Verification items for the finished model (mm, model axes). A direction names the side the tool comes from. Give positions to 0.01 mm unless a question says otherwise; leave off trailing zeros. Write each loop counter-clockwise with the first axis right and the second up, starting at its lowest first coordinate (ties: lowest second). Pieces come first, ordered by that corner, then holes. Notation, with made-up numbers: M 2.25,-10 L 50.25,-10 A34 cw 50.25,23 Z; hole C 30.5,-33.5 d2. An arc over 180 degrees is marked long. Answer as a JSON object with one key per item and string values.
```python
from build123d import *

# Parameters (mm, degrees)
SKETCH_2_R               = 6.25
CUT_EXTRUDE_1_DEPTH      = 140.896390232
PATTERN_CIRCULAR_1_COUNT = 6
SKETCH_3_R               = 27.5
CUT_EXTRUDE_2_DEPTH      = 140.896390232
CUT_EXTRUDE_START        = -15
CUT_EXTRUDE_3_DEPTH      = 15
PATTERN_CIRCULAR_2_COUNT = 6
PATTERN_CIRCULAR_3_COUNT = 6


with BuildPart() as part:
    # 草图1 → 旋转1 (revolve)
    with BuildSketch(Plane.XY, mode=Mode.PRIVATE) as revolve_1_sk:
        Polygon((0, 0), (0, 95), (30, 95), (30, 50), (39, 50), (39, 35), (30, 35), (30, 0), align=None)
    revolve(revolve_1_sk.sketch.rotate(Axis((0, 0, 0), (1, 0, 0)), 90), axis=Axis((0, 0, 0), (1, 0, 0)))

    # 草图2 → 切除-拉伸1 (cut, through all)
    with BuildSketch(Plane.ZY):
        with Locations((0, 80)):
            Circle(SKETCH_2_R)
    cut_extrude_1 = extrude(amount=-CUT_EXTRUDE_1_DEPTH, mode=Mode.SUBTRACT)

    # 阵列(圆周)1: 切除-拉伸1 ×6 about axis
    pattern_circular_1_axis = Axis((0, 0, 0), (1, 0, 0))
    for i in range(1, PATTERN_CIRCULAR_1_COUNT):
        add(cut_extrude_1.rotate(pattern_circular_1_axis, i * 360 / PATTERN_CIRCULAR_1_COUNT), mode=Mode.SUBTRACT)

    # 草图3 → 切除-拉伸2 (cut, through all)
    with BuildSketch(Plane.ZY):
        Circle(SKETCH_3_R)
    extrude(amount=-CUT_EXTRUDE_2_DEPTH, mode=Mode.SUBTRACT)

    # 草图6 → 切除-拉伸3 (cut)
    with BuildSketch(Plane.ZY.offset(CUT_EXTRUDE_START)):
        with BuildLine():
            Line((-16, 80), (-16, 93.642938869))
            ThreePointArc((-16, 93.642938869), (0, 95), (16, 93.642938869))
            Line((16, 93.642938869), (16, 80))
            ThreePointArc((16, 80), (0, 64), (-16, 80))
        make_face()
    cut_extrude_3 = extrude(amount=CUT_EXTRUDE_3_DEPTH, mode=Mode.SUBTRACT)

    # 阵列(圆周)2: 切除-拉伸3 ×6 about axis
    pattern_circular_2_axis = Axis((0, 0, 0), (1, 0, 0))
    for i in range(1, PATTERN_CIRCULAR_2_COUNT):
        add(cut_extrude_3.rotate(pattern_circular_2_axis, i * 360 / PATTERN_CIRCULAR_2_COUNT), mode=Mode.SUBTRACT)

    # 草图8 → M12 螺纹孔1 (revolve, cut)
    with BuildSketch(Plane(origin=(0, 69.282032303, 40), x_dir=(0, 0, 1), z_dir=(0, 1, 0))):
        Polygon((0, 0), (0, 21.064389157), (5.1, 18), (5.1, 0), align=None)
    hole_wizard_m12_1 = revolve(axis=Axis((-6.35, 69.282032303, 40), (1, 0, 0)), mode=Mode.SUBTRACT)

    # 阵列(圆周)3: M12 螺纹孔1 ×6 about axis
    pattern_circular_3_axis = Axis((0, 0, 0), (1, 0, 0))
    for i in range(1, PATTERN_CIRCULAR_3_COUNT):
        add(hole_wizard_m12_1.rotate(pattern_circular_3_axis, i * 360 / PATTERN_CIRCULAR_3_COUNT), mode=Mode.SUBTRACT)


solid = part.part
```
1) Section check C-C on z = 22.5. Record the boundary of the cut face in (x, y).
Completed:
{"outline": "M 0,-92.3 L 30,-92.3 L 30,-44.65 L 39,-44.65 L 39,-26.81 L 30,-26.81 L 30,-15.81 L 0,-15.81 Z; M 0,15.81 L 30,15.81 L 30,26.81 L 39,26.81 L 39,44.65 L 30,44.65 L 30,92.3 L 0,92.3 Z"}
2) Go/stop test with flat-tipped pins: pin 1 (18 mm diameter, centred on y = -45, z = -62.5, fed in from -X); pin 2 (15 mm diameter, centred on x = 7, y = -83.5, fed in from -Z); pin 3 (4 mm diameter, centred on x = 18.5, y = -29.5, fed in from +Z); pin 4 (1.5 mm diameter, centred on x = 29, z = 48, fed in from +Y). Record where each tip stops, or that it passes through.
Completed:
{"pin 1": "stops at x = 0", "pin 2": "stops at z = -57", "pin 3": "stops at z = 90.93", "pin 4": "stops at y = 82.42"}
3) Access from +Z, -Z, +X, -X, +Y, -Y to the whole of each face (thin tool, end or side, straight path). Record for faces 5 (the face through (7.6, -29.6, -83.27)), 6 (the face through (7.605, -57.315, 67.272)), 7 (the face through (30, 18, -21)), 8 (the face through (15, -43, 75)).
Completed:
{"face 5": "-X, -Y", "face 6": "+Z, -X", "face 7": "+X", "face 8": "-X"}
4) Release check for a two-part mould opening along Y. For faces 1 (the face through (15, 87, 0)), 2 (the face through (15, -43, -75)), 3 (the face through (7.6, 32.31, -55.25)), 4 (the face through (7.6, 29.51, -83.11)) record: pulls with the +Y half, pulls with the -Y half, needs draft (parallel to the pull), parting line crosses it, or undercut.
Completed:
{"face 1": "needs draft", "face 2": "undercut", "face 3": "undercut", "face 4": "pulls with the +Y half"}
5) Section check A-A on z = 0. Record the boundary of the cut face in (x, y).
Completed:
{"outline": "M 0,-64 L 15,-64 L 15,-73.75 L 30,-73.75 L 30,-50 L 39,-50 L 39,-35 L 30,-35 L 30,-27.5 L 0,-27.5 Z; M 0,27.5 L 30,27.5 L 30,35 L 39,35 L 39,50 L 30,50 L 30,73.75 L 15,73.75 L 15,64 L 0,64 Z; M 15,-95 L 30,-95 L 30,-86.25 L 15,-86.25 Z; M 15,86.25 L 30,86.25 L 30,95 L 15,95 Z"}
6) Section check D-D on x = 5. Count the separate pieces of the cut face and the enclosed holes in it, and give its area (3 significant figures).
Completed:
{"separate pieces": "1", "enclosed holes": "7", "area": "20,300 mm2"}
7) Section check B-B on y = -40. Record the boundary of the cut face in (x, z), and give its area (3 significant figures).
Completed:
{"outline": "M 0,-53.28 L 15,-53.28 L 15,-63.03 L 30,-63.03 L 30,-30 L 39,-30 L 39,30 L 30,30 L 30,63.03 L 15,63.03 L 15,53.28 L 0,53.28 Z; M 15,-86.17 L 30,-86.17 L 30,-75.53 L 15,-75.53 Z; M 15,75.53 L 30,75.53 L 30,86.17 L 15,86.17 Z", "area": "4,350 mm2"}
8) Thickness scan on L1, parallel to Z at x = 9.5, y = -73.5; L2, parallel to Y at x = 22, z = -74; L3, parallel to X at y = -59.5, z = 60. Record the ranges inside material, lowest first.
Completed:
{"L1": "z = -60.19 to -42.87, -37.13 to -14.62, 14.62 to 37.13, 42.87 to 60.19", "L2": "y = -59.57 to -44.1, -35.9 to 35.9, 44.1 to 59.57", "L3": "x = 0 to 30"}
